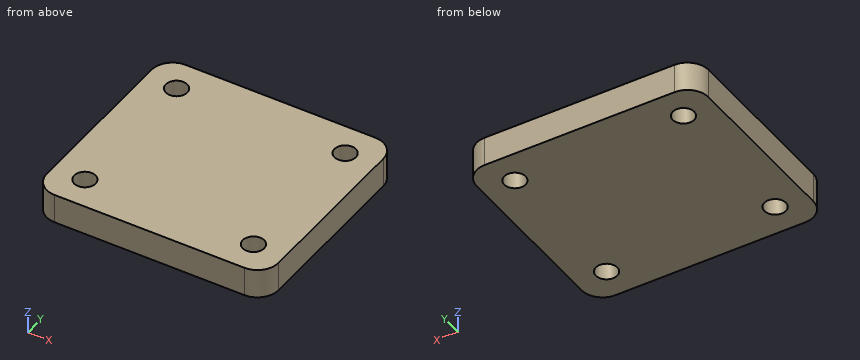
from build123d import *

# Parameters (mm, degrees)
EXTRUDE_1_DEPTH         = 14
HOLE_WIZARD_M12_1_D     = 10.2
HOLE_WIZARD_M12_1_DEPTH = 29.25
HOLE_WIZARD_M12_1_TIP   = 3.064389157


with BuildPart() as part:
    # 草图1 → 凸台-拉伸1 (new body)
    with BuildSketch(Plane.XY):
        with BuildLine():
            Line((10, 0), (100, 0))
            ThreePointArc((100, 0), (107.071067812, 2.928932188), (110, 10))
            Line((110, 10), (110, 90))
            ThreePointArc((110, 90), (107.071067812, 97.071067812), (100, 100))
            Line((100, 100), (10, 100))
            ThreePointArc((10, 100), (2.928932188, 97.071067812), (0, 90))
            Line((0, 90), (0, 10))
            ThreePointArc((0, 10), (2.928932188, 2.928932188), (10, 0))
        make_face()
    extrude(amount=EXTRUDE_1_DEPTH)

    # M12 螺纹孔1
    with Locations(Plane(origin=(15, 85, 14), x_dir=(1, 0, 0), z_dir=(0, 0, 1))):
        with Locations((0, 0), (80, 0), (80, -70), (0, -70)):
            Hole(HOLE_WIZARD_M12_1_D / 2, depth=HOLE_WIZARD_M12_1_DEPTH)
            with Locations((0, 0, -(HOLE_WIZARD_M12_1_DEPTH + HOLE_WIZARD_M12_1_TIP / 2))):  # 118° drill point
                Cone(0, HOLE_WIZARD_M12_1_D / 2, HOLE_WIZARD_M12_1_TIP, mode=Mode.SUBTRACT)


solid = part.part
Here's how the part is built. I have some questions about the finished solid (model axes, mm). Give positions to 0.01 mm unless a question says otherwise; leave off trailing zeros. Loops run counter-clockwise (first coordinate to the right, second up) from the corner with the lowest first, then second, coordinate; pieces in that order, holes last. Notation, with made-up numbers: (43, 22) -> (97, 22) arc R24 cw to (97, 38) -> close; hole circle Ø7 at (25.25, -21). An arc over 180 degrees is marked (long way). Answer as a JSON object with one key per item and string values. Group by question number.
Item 1: Imagine slicing it at C-C on z = 9.5. Write out the boundary of the cut face in (x, y), then the cut area to 3 significant figures.
Item 2: Imagine slicing it at A-A on x = 15. Write out the boundary of the cut face in (y, z), then the cut area to 3 significant figures.
Item 3: Will this pin go through, and if not, where does the flat tip stop? pin 1 (16.5 mm diameter, centred on x = 95, y = 15, fed in from -Z).
Item 4: Imagine slicing it at B-B on y = 15. Write out the boundary of the cut face in (x, z).
Item 5: I need wall thicknesses on L1, parallel to Y at x = 15, z = 9.75; L2, parallel to X at y = 80.5, z = 7; L3, parallel to X at y = 7, z = 11.75. Which ranges of each line are inside material? Lowest first, please.
Answer list:
{
 "1": {"outline": "(0, 10) arc R10 ccw to (10, 0) -> (100, 0) arc R10 ccw to (110, 10) -> (110, 90) arc R10 ccw to (100, 100) -> (10, 100) arc R10 ccw to (0, 90) -> close; hole circle Ø10.2 at (15, 15); hole circle Ø10.2 at (15, 85); hole circle Ø10.2 at (95, 15); hole circle Ø10.2 at (95, 85)", "area": "10,600 mm2"},
 "2": {"outline": "(0, 0) -> (9.9, 0) -> (9.9, 14) -> (0, 14) -> close; (20.1, 0) -> (79.9, 0) -> (79.9, 14) -> (20.1, 14) -> close; (90.1, 0) -> (100, 0) -> (100, 14) -> (90.1, 14) -> close", "area": "1,110 mm2"},
 "3": {"pin 1": "stops at z = 0"},
 "4": {"outline": "(0, 0) -> (9.9, 0) -> (9.9, 14) -> (0, 14) -> close; (20.1, 0) -> (89.9, 0) -> (89.9, 14) -> (20.1, 14) -> close; (100.1, 0) -> (110, 0) -> (110, 14) -> (100.1, 14) -> close"},
 "5": {"L1": "y = 0 to 9.9, 20.1 to 79.9, 90.1 to 100", "L2": "x = 0 to 12.6, 17.4 to 92.6, 97.4 to 110", "L3": "x = 0.46 to 109.54"}
}
